```python
from build123d import *

# Parameters (mm, degrees)
SKETCH1_W           = 40
SKETCH1_H           = 40
BOSS_EXTRUDE1_DEPTH = 10
FILLET1_R           = 20


with BuildPart() as part:
    # Sketch1 → Boss-Extrude1 (new body)
    with BuildSketch(Plane.XY):
        with Locations((20, 20)):
            Rectangle(SKETCH1_W, SKETCH1_H)
    extrude(amount=BOSS_EXTRUDE1_DEPTH)

    # Fillet1
    fillet1_edges = [part.edges().sort_by_distance(p)[0] for p in [
        (0, 40, 5),
    ]]
    fillet(fillet1_edges, radius=FILLET1_R)


solid = part.part
```
The model under review builds one solid part; all positions refer to its coordinate system, in mm. Round coordinates to 2 decimals unless told otherwise and drop trailing zeros. Loops run counter-clockwise (first coordinate to the right, second up) from the corner with the lowest first, then second, coordinate; pieces in that order, holes last.
Item 1: Take a section at A-A (z = 1.75). Write out the cut boundary in (x, y).
Determined:
outline: (0, 0) - (40, 0) - (40, 40) - (20, 40) arc R20 ccw to (0, 20) - close
Item 2: Take a section at C-C (x = 5.5). Write out the cut boundary in (y, z).
Determined:
outline: (0, 0) - (33.77, 0) - (33.77, 10) - (0, 10) - close
Item 3: For line 1 (X direction, y = 20.5, z = 9.25); line 2 (X direction, y = 36, z = 1); line 3 (Y direction, x = 16, z = 7.25), list the stretches that pass through material, from the lowest coordinate up.
Determined:
line 1: x = 0.01 to 40
line 2: x = 8 to 40
line 3: y = 0 to 39.6
Item 4: Take a section at B-B (y = 36.5). Write out the cut boundary in (x, z).
Determined:
outline: (8.7, 0) - (40, 0) - (40, 10) - (8.7, 10) - close
Item 5: Clearance check with flat-ended pins moving along their axes: pin 1 Ø2 at (x, z) = (10.5, 4.5) entering from +Y; pin 2 Ø2 at (y, z) = (26, 4) entering from -X. State where each tip first meets the part, or that it passes through.
Determined:
pin 1: stops at y = 38.1
pin 2: stops at x = 0.64
Item 6: Mouldability with a two-part tool opening along X and no side actions: class faces 1 (the face through (20, 0, 5)), 2 (the face through (40, 20, 5)), 3 (the face through (5.703, 33.986, 5.07)) as released by +X, released by -X, zero draft, split by the parting line, or undercut.
Determined:
face 1: zero draft
face 2: released by +X
face 3: released by -X
